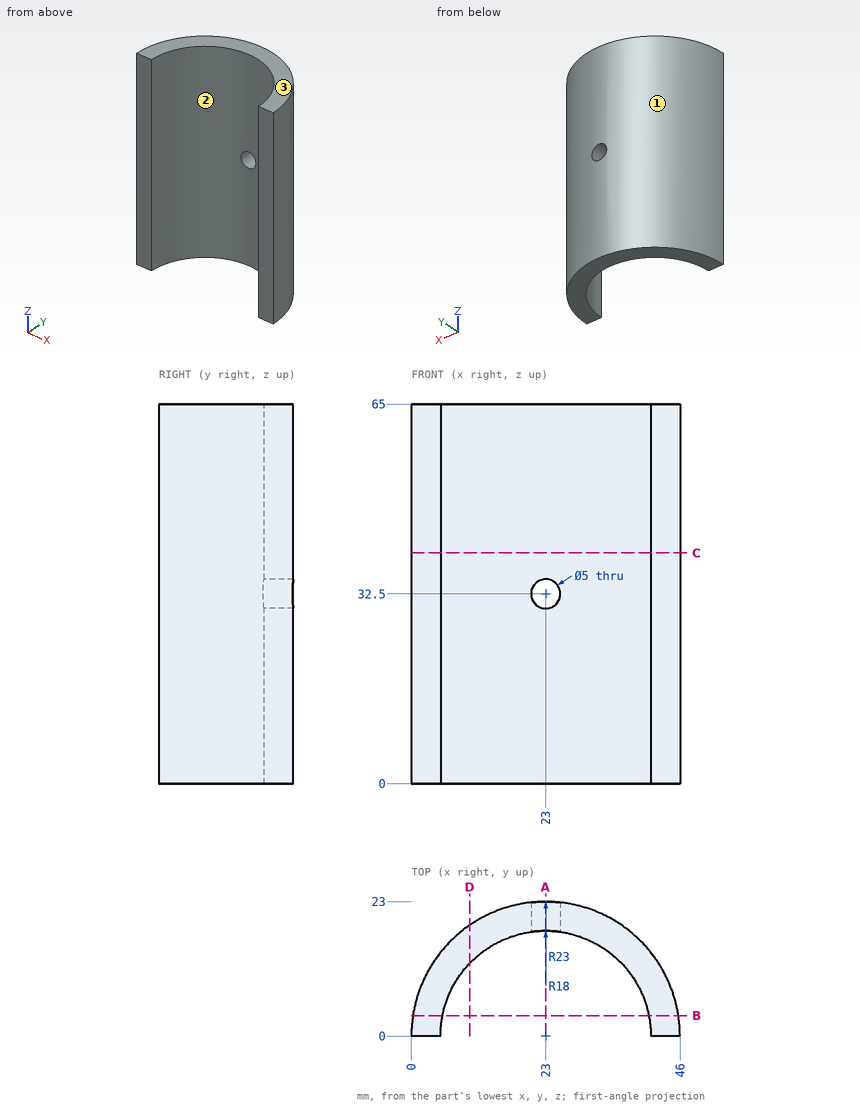
Geometry: see drawing. Coordinates: mm, zero at the bounding-box minimum. Coordinates: 2 decimals unless noted, no trailing zeros. Loops run counter-clockwise (first coordinate to the right, second up) from the corner with the lowest first, then second, coordinate; pieces in that order, holes last. Notation, with made-up numbers: (12.25, -19) - (56.25, -19) arc R36 cw to (56.25, 19) - close; hole circle Ø9 at (24, 63). An arc over 180 degrees is marked (long way). Answer as CSV lines item,"result".
1. Ray query, line 1 (Z direction, x = 23, y = 21.2); line 2 (X direction, y = 6.5, z = 22); line 3 (X direction, y = 1.25, z = 56). Return the intervals inside material, ascending.
Established:
line 1,"z = 0 to 30, 35 to 65"
line 2,"x = 0.94 to 6.21, 39.79 to 45.06"
line 3,"x = 0.03 to 5.04, 40.96 to 45.97"
2. Section D-D (x = 10). Return loops of the section in (y, z).
Established:
outline,"(12.45, 0) - (18.97, 0) - (18.97, 65) - (12.45, 65) - close"
3. Section B-B (y = 3.5). Return loops of the section in (x, z), then the cut area to 3 significant figures.
Established:
outline,"(0.27, 0) - (5.34, 0) - (5.34, 65) - (0.27, 65) - close; (40.66, 0) - (45.73, 0) - (45.73, 65) - (40.66, 65) - close"
area,"660 mm2"
4. Section A-A (x = 23). Return loops of the section in (y, z).
Established:
outline,"(18, 0) - (23, 0) - (23, 30) - (18, 30) - close; (18, 35) - (23, 35) - (23, 65) - (18, 65) - close"
5. Contact query for flat-ended pins moving along their axis: pin 1 (3 mm diameter, centred on x = 15.5, z = 30, fed in from +Y); pin 2 (1 mm diameter, centred on y = 18, z = 26.5, fed in from -X); pin 3 (5 mm diameter, centred on x = 41, z = 20, fed in from +Y); pin 4 (4.5 mm diameter, centred on x = 23, z = 32.5, fed in from -Y). Output: stop coordinate, or through.
Established:
pin 1,"stops at y = 22.2"
pin 2,"stops at x = 8.08"
pin 3,"stops at y = 16.99"
pin 4,"passes through"
6. Mould query, pull axis X, two halves, no side actions, for the marked faces 1, 2 and 3. Classes: released by +X, released by -X, zero draft, split by the parting line, or undercut.
Established:
face 1,"split by the parting line"
face 2,"undercut"
face 3,"zero draft"
7. Section C-C (z = 39.5). Return loops of the section in (x, y), then the cut area to 3 significant figures.
Established:
outline,"(0, 0) - (5, 0) arc R18 cw to (41, 0) - (46, 0) arc R23 ccw to start"
area,"322 mm2"
